Source: CAD feature listing. Evaluate the final solid. Frame: model axes, mm. Face numbers are marked on the shaded views. A direction names the side the tool comes from. Round coordinates to 2 decimals unless told otherwise and drop trailing zeros. Write each loop counter-clockwise with the first axis right and the second up, starting at its lowest first coordinate (ties: lowest second). Pieces come first, ordered by that corner, then holes. Notation, with made-up numbers: (51, -23.5) - (73, -23.5) arc R24 ccw to (73, -4.5) - close; hole circle Ø8 at (33, 89). An arc over 180 degrees is marked (long way). Write item = value, one per line. Start each with the question number.
```python
from build123d import *

# Parameters (mm, degrees)
EXTRUDE_1_DEPTH = 50


with BuildPart() as part:
    # 草图1 → 凸台-拉伸1 (new body)
    with BuildSketch(Plane.XY):
        with BuildLine():
            Line((-225, 42.5), (225, 42.5))
            ThreePointArc((225, 42.5), (267.5, 0), (225, -42.5))
            Line((225, -42.5), (-225, -42.5))
            ThreePointArc((-225, -42.5), (-267.5, 0), (-225, 42.5))
        make_face()
        with BuildLine():
            Line((-225, 37.5), (225, 37.5))
            ThreePointArc((225, 37.5), (262.5, 0), (225, -37.5))
            Line((225, -37.5), (-225, -37.5))
            ThreePointArc((-225, -37.5), (-262.5, 0), (-225, 37.5))
        make_face(mode=Mode.SUBTRACT)
    extrude(amount=EXTRUDE_1_DEPTH)


solid = part.part
```
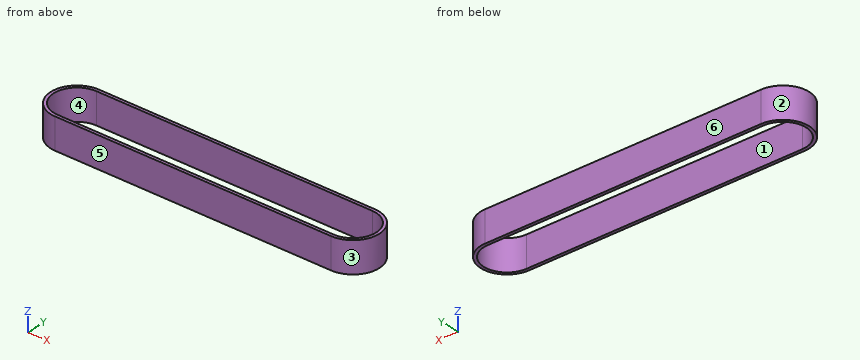
(1) Contact query for a flat-ended pin moving along its axis: P1, Ø1.5, axis at y = 1.5, z = 40.5, coming from the -X side. Output: stop coordinate, or through.
(2) Section C-C (z = 9.5). Return the cut outline in (x, y).
(3) Ray query, L1, parallel to Y at x = -172.5, z = 26.5; L2, parallel to X at y = 27.5, z = 33.5; L3, parallel to X at y = -25.5, z = 19. Return the intervals inside material, ascending. Write a range as from..to.
(4) Reachability of the marked faces 1 and 2 from +Z, -Z, +X, -X, +Y, -Y: full face, straight path, thin tool, end or side. Return the list, or none.
(5) Pull-direction query (Y, two-part tool) for the marked faces 3, 4, 5 and 6; classes: +Y half, -Y half, draft (parallel to the pull), parting line (faces both ways), or undercut.
(6) Section A-A (x = 106.5). Return the cut outline in (y, z).
(7) Section B-B (y = 0). Return the cut outline in (x, z).
Solution:
q1.P1 = -267.49
q2.outline = (-225, -42.5) - (225, -42.5) arc R42.5 ccw to (225, 42.5) - (-225, 42.5) arc R42.5 ccw to start; hole (-225, -37.5) - (225, -37.5) arc R37.5 ccw to (225, 37.5) - (-225, 37.5) arc R37.5 ccw to start
q3.L1 = -42.5..-37.5, 37.5..42.5
q3.L2 = -257.4..-250.5, 250.5..257.4
q3.L3 = -259..-252.5, 252.5..259
q4.face_1 = +Z, -Z
q4.face_2 = +Z, -Z, -X
q5.face_3 = parting line
q5.face_4 = undercut
q5.face_5 = -Y half
q5.face_6 = +Y half
q6.outline = (-42.5, 0) - (-37.5, 0) - (-37.5, 50) - (-42.5, 50) - close; (37.5, 0) - (42.5, 0) - (42.5, 50) - (37.5, 50) - close
q7.outline = (-267.5, 0) - (-262.5, 0) - (-262.5, 50) - (-267.5, 50) - close; (262.5, 0) - (267.5, 0) - (267.5, 50) - (262.5, 50) - close
